from build123d import *

# Parameters (mm, degrees)
SKETCH1_R                  = 105
BOSS_EXTRUDE1_DEPTH        = 15
F_14_0_14_DIAMETER_HOLE1_D = 14


with BuildPart() as part:
    # Sketch1 → Boss-Extrude1 (new body)
    with BuildSketch(Plane(origin=(0, 0, 0), x_dir=(1, 0, 0), z_dir=(0, 1, 0))):
        with Locations(Location((0, 0, 0), (0, 0, 270))):
            Circle(SKETCH1_R)
    extrude(amount=BOSS_EXTRUDE1_DEPTH)

    # Ø14.0 (14) Diameter Hole1 (through all)
    with Locations(Plane(origin=(0, 15, 0), x_dir=(1, 0, 0), z_dir=(0, 1, 0))):
        with Locations((0, 90), (90, 0), (0, -90), (-90, 0)):
            Hole(F_14_0_14_DIAMETER_HOLE1_D / 2)


solid = part.part
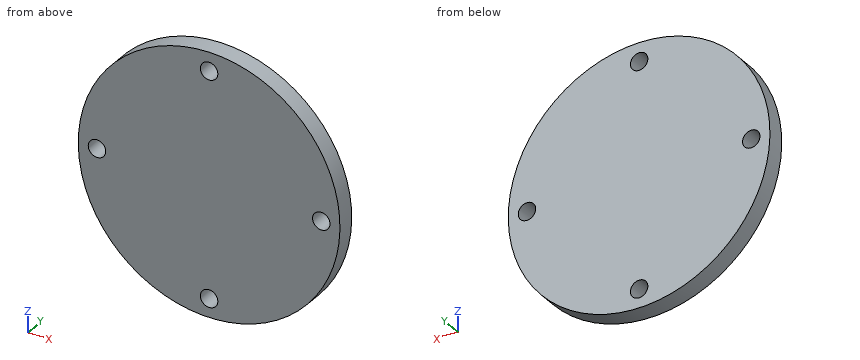
Read the model definition and answer for the solid it produces. Units are mm, in the model's axes. Give positions to 0.01 mm unless a question says otherwise; leave off trailing zeros. Write each loop counter-clockwise with the first axis right and the second up, starting at its lowest first coordinate (ties: lowest second). Pieces come first, ordered by that corner, then holes. Notation, with made-up numbers: (-23, 53) -> (1, 53) arc R18 ccw to (1, 71) -> close; hole circle Ø1 at (-2, 44.5). An arc over 180 degrees is marked (long way). Answer as a JSON object with one key per item and string values. Group by question number.
1) Find section D-D (x = 90). Write down the section's boundary in (y, z), and give its area (3 significant figures).
2) Consider L1, parallel to Z at x = -90, y = 5.5; L2, parallel to Z at x = 16, y = 3.75. Determine where each line is inside the solid, lowest interval first. Write a range as from..to.
3) Find section C-C (y = 12). Write down the section's boundary in (x, z), and give its area (3 significant figures).
4) Find section B-B (x = 0). Write down the section's boundary in (y, z).
5) Find section A-A (z = 0). Write down the section's boundary in (x, y).
6) Each of these flat-tipped pins is pushed along its axis until it touches: P1, Ø2, axis at y = 2.5, z = -69, coming from the -X side; P2, Ø1, axis at y = 2, z = 5, coming from the -X side; P3, Ø1.5, axis at y = 13, z = -19.5, coming from the -X side. Where does it stop, or does it pass through?
Values follow:
{
 "1": {"outline": "(0, -54.08) -> (15, -54.08) -> (15, -7) -> (0, -7) -> close; (0, 7) -> (15, 7) -> (15, 54.08) -> (0, 54.08) -> close", "area": "1,410 mm2"},
 "2": {"L1": "z = -54.08..-7, 7..54.08", "L2": "z = -103.77..103.77"},
 "3": {"outline": "circle Ø210 at (0, 0); hole circle Ø14 at (-90, 0); hole circle Ø14 at (0, -90); hole circle Ø14 at (0, 90); hole circle Ø14 at (90, 0)", "area": "34,000 mm2"},
 "4": {"outline": "(0, -105) -> (15, -105) -> (15, -97) -> (0, -97) -> close; (0, -83) -> (15, -83) -> (15, 83) -> (0, 83) -> close; (0, 97) -> (15, 97) -> (15, 105) -> (0, 105) -> close"},
 "5": {"outline": "(-105, 0) -> (-97, 0) -> (-97, 15) -> (-105, 15) -> close; (-83, 0) -> (83, 0) -> (83, 15) -> (-83, 15) -> close; (97, 0) -> (105, 0) -> (105, 15) -> (97, 15) -> close"},
 "6": {"P1": "stops at x = -80.01", "P2": "stops at x = -104.9", "P3": "stops at x = -103.31"}
}
